Geometry: final body of the model. Coordinates: model frame, mm. A direction names the side the tool comes from. Coordinates: 2 decimals unless noted, no trailing zeros. Write each loop counter-clockwise with the first axis right and the second up, starting at its lowest first coordinate (ties: lowest second). Pieces come first, ordered by that corner, then holes.
from build123d import *

# Parameters (mm, degrees)
SKETCH_1_W                = 150
SKETCH_1_H                = 150
EXTRUDE_1_DEPTH           = 16
CUT_EXTRUDE_1_DEPTH       = 108.266024444
HOLE_WIZARD_1_D           = 9
HOLE_WIZARD_1_DEPTH       = 29.25
HOLE_WIZARD_1_CBORE_D     = 15
HOLE_WIZARD_1_CBORE_DEPTH = 9
HOLE_WIZARD_1_TIP         = 2.703872786
HOLE_WIZARD_2_D           = 9
HOLE_WIZARD_2_DEPTH       = 29.25
HOLE_WIZARD_2_CBORE_D     = 15
HOLE_WIZARD_2_CBORE_DEPTH = 9
HOLE_WIZARD_2_TIP         = 2.703872786
CHAMFER_1_SIZE            = 10


with BuildPart() as part:
    # 草图1 → 凸台-拉伸1 (new body)
    with BuildSketch(Plane(origin=(0, 0, 0), x_dir=(0, 0, -1), z_dir=(1, 0, 0))):
        Rectangle(SKETCH_1_W, SKETCH_1_H)
    extrude(amount=EXTRUDE_1_DEPTH)

    # 草图3 → 切除-拉伸1 (cut, through all)
    with BuildSketch(Plane(origin=(16, 0, 0), x_dir=(0, 0, -1), z_dir=(1, 0, 0))):
        with BuildLine():
            Line((-37.253402877, 35), (-37.253402877, -65))
            ThreePointArc((-37.253402877, -65), (-43.753402877, -71.5), (-50.253402877, -65))
            Line((-50.253402877, -65), (-50.253402877, 35))
            ThreePointArc((-50.253402877, 35), (-43.753402877, 41.5), (-37.253402877, 35))
        make_face()
        with BuildLine():
            Line((50.253402877, 35), (50.253402877, -65))
            ThreePointArc((50.253402877, -65), (43.753402877, -71.5), (37.253402877, -65))
            Line((37.253402877, -65), (37.253402877, 35))
            ThreePointArc((37.253402877, 35), (43.753402877, 41.5), (50.253402877, 35))
        make_face()
    extrude(amount=-CUT_EXTRUDE_1_DEPTH, mode=Mode.SUBTRACT)

    # 打孔尺寸(%根据)内六角圆柱头螺钉的类型1
    with Locations(Plane.ZY):
        with Locations((-50, 67), (0, 67), (50, 67)):
            CounterBoreHole(HOLE_WIZARD_1_D / 2, HOLE_WIZARD_1_CBORE_D / 2, HOLE_WIZARD_1_CBORE_DEPTH, depth=HOLE_WIZARD_1_DEPTH)
            with Locations((0, 0, -(HOLE_WIZARD_1_DEPTH + HOLE_WIZARD_1_TIP / 2))):  # 118° drill point
                Cone(0, HOLE_WIZARD_1_D / 2, HOLE_WIZARD_1_TIP, mode=Mode.SUBTRACT)

    # 打孔尺寸(%根据)内六角圆柱头螺钉的类型2
    with Locations(Plane.ZY):
        with Locations((-60, 39), (-60, -11), (60, 39), (60, -11)):
            CounterBoreHole(HOLE_WIZARD_2_D / 2, HOLE_WIZARD_2_CBORE_D / 2, HOLE_WIZARD_2_CBORE_DEPTH, depth=HOLE_WIZARD_2_DEPTH)
            with Locations((0, 0, -(HOLE_WIZARD_2_DEPTH + HOLE_WIZARD_2_TIP / 2))):  # 118° drill point
                Cone(0, HOLE_WIZARD_2_D / 2, HOLE_WIZARD_2_TIP, mode=Mode.SUBTRACT)

    # 倒角1
    chamfer_1_edges = [part.edges().sort_by_distance(p)[0] for p in [
        (8, -75, -75),
        (8, -75, 75),
    ]]
    chamfer(chamfer_1_edges, length=CHAMFER_1_SIZE)


solid = part.part
Item 1: Section A-A, the plane y = -39. Output: boundary loops of the cut face in (x, z).
Derived:
outline: (0, -75) - (16, -75) - (16, -50.25) - (0, -50.25) - close; (0, -37.25) - (16, -37.25) - (16, 37.25) - (0, 37.25) - close; (0, 50.25) - (16, 50.25) - (16, 75) - (0, 75) - close
Item 2: Set-up query: faces 5 (the flat face through (16, 1, 1)), 6 (the cylindrical face through (8.1, -71.5, -43.9)), 7 (the flat face through (9, 67, 5)). Return all of +Z, -Z, +X, -X, +Y, -Y with unobstructed straight access to the full face (end or side cutting, diameter ignored); none if empty.
Derived:
face 5: +Z, -Z, +X, +Y, -Y
face 6: +X, -X
face 7: -X
Item 3: Section B-B, the plane z = 0. Output: boundary loops of the cut face in (x, y), plus the area to 3 significant figures.
Derived:
outline: (0, -75) - (16, -75) - (16, 62.5) - (9, 62.5) - (9, 59.5) - (0, 59.5) - close; (0, 74.5) - (9, 74.5) - (9, 71.5) - (16, 71.5) - (16, 75) - (0, 75) - close
area: 2,200 mm2
Item 4: Section C-C, the plane x = 6.5. State how many separate pieces and enclosed holes the cut face has, plus the area to 3 significant figures.
Derived:
separate pieces: 1
enclosed holes: 9
area: 18,300 mm2
Item 5: Section D-D, the plane y = 67. Output: boundary loops of the cut face in (x, z).
Derived:
outline: (0, -75) - (16, -75) - (16, -54.5) - (9, -54.5) - (9, -57.5) - (0, -57.5) - close; (0, -42.5) - (9, -42.5) - (9, -45.5) - (16, -45.5) - (16, -4.5) - (9, -4.5) - (9, -7.5) - (0, -7.5) - close; (0, 7.5) - (9, 7.5) - (9, 4.5) - (16, 4.5) - (16, 45.5) - (9, 45.5) - (9, 42.5) - (0, 42.5) - close; (0, 57.5) - (9, 57.5) - (9, 54.5) - (16, 54.5) - (16, 75) - (0, 75) - close
Item 6: Pull-direction query (Y, two-part tool) for faces 1 (the flat face through (8, 75, 1)), 2 (the flat face through (8, -70, -70)), 3 (the flat face through (9, 62, -50)), 4 (the flat face through (0, 1, 1)); classes: released by +Y, released by -Y, zero draft, split by the parting line, or undercut.
Derived:
face 1: released by +Y
face 2: released by -Y
face 3: undercut
face 4: zero draft
Item 7: Pin query (flat end, axial travel): pin 1 (12 mm diameter, centred on y = -11, z = 60, fed in from -X). Return the tip coordinate at first contact, or that it passes through.
Derived:
pin 1: stops at x = 9
Item 8: Material intervals for probe 1 along Z at (x, y) = (7.75, 61); probe 2 along Y at (x, z) = (12, -60); probe 3 along Z at (x, y) = (14, -50.5), sorted ascending.
Derived:
probe 1: z = -75 to -54.5, -45.5 to -4.5, 4.5 to 45.5, 54.5 to 75
probe 2: y = -75 to -15.5, -6.5 to 34.5, 43.5 to 75
probe 3: z = -75 to -50.25, -37.25 to 37.25, 50.25 to 75
